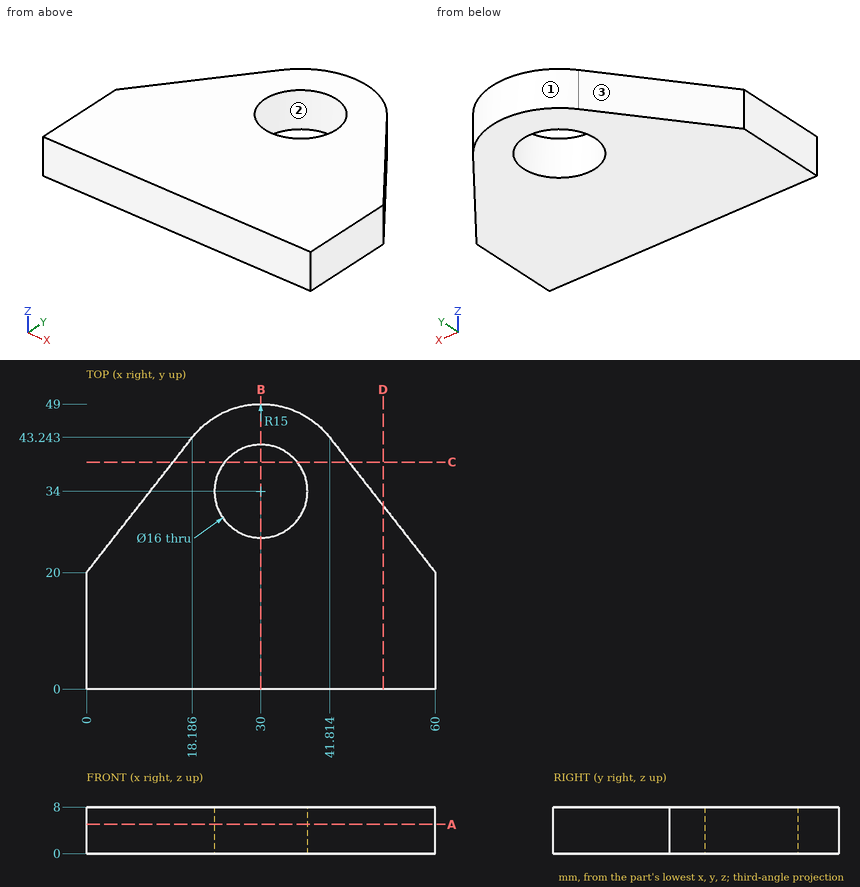
Could you check a few things on this drawing? It's one solid part, dimensions in mm from its lowest x, y, z. Give positions to 0.01 mm unless a question says otherwise; leave off trailing zeros. Write each loop counter-clockwise with the first axis right and the second up, starting at its lowest first coordinate (ties: lowest second). Pieces come first, ordered by that corner, then holes. Notation, with made-up numbers: M 20,3 L 62,3 A31 ccw 62,29 Z; hole C 62,60.5 d4. An arc over 180 degrees is marked long. Put each result on its own line as item: value. Start each with the question number.
Item 1: I need wall thicknesses on L1, parallel to Y at x = 30, z = 6.5; L2, parallel to X at y = 27, z = 4 (1 decimal); L3, parallel to X at y = 35, z = 2.25 (1 decimal). Which ranges of each line are inside material? Lowest first, please. Write a range as from..to.
Item 2: If we section it at A-A, the plane z = 5: Write out the boundary of the cut face in (x, y), then the cut area to 3 significant figures.
Item 3: If we section it at C-C, the plane y = 39: Write out the boundary of the cut face in (x, z) (1 decimal).
Item 4: Will these pins go through, and if not, where does the flat tip stop? pin 1 (2 mm diameter, centred on y = 21.5, z = 1.5, fed in from +X); pin 2 (4 mm diameter, centred on x = 9, z = 5.5, fed in from +Y); pin 3 (1 mm diameter, centred on x = 33, z = 1.5, fed in from +Y).
Item 5: Thinking about a two-plate mould opening in X: for the marked faces 1, 2 and 3, which applies, +X half, -X half, draft (parallel to the pull), parting line (faces both ways), or undercut?
Item 6: If we section it at B-B, the plane x = 30: Write out the boundary of the cut face in (y, z).
Item 7: If we section it at D-D, the plane x = 51: Write out the boundary of the cut face in (y, z), then the cut area to 3 significant figures.
Values:
1. L1: 0..26, 42..49
1. L2: 5.5..26.1, 33.9..54.5
1. L3: 11.7..22.1, 37.9..48.3
2. outline: M 0,0 L 60,0 L 60,20 L 41.81,43.24 A15 ccw 18.19,43.24 L 0,20 Z; hole C 30,34 d16
2. area: 2,070 mm²
3. outline: M 14.9,0 L 23.8,0 L 23.8,8 L 14.9,8 Z; M 36.2,0 L 45.1,0 L 45.1,8 L 36.2,8 Z
4. pin 1: x = 59.61
4. pin 2: y = 34.06
4. pin 3: y = 48.79
5. face 1: parting line
5. face 2: undercut
5. face 3: -X half
6. outline: M 0,0 L 26,0 L 26,8 L 0,8 Z; M 42,0 L 49,0 L 49,8 L 42,8 Z
7. outline: M 0,0 L 31.5,0 L 31.5,8 L 0,8 Z
7. area: 252 mm²
